```python
from build123d import *

# Parameters (mm, degrees)
SKETCH_1_R          = 2
EXTRUDE_1_DEPTH     = 10
SKETCH_2_R          = 1.5
CUT_EXTRUDE_1_DEPTH = 6
SKETCH_3_W          = 5
SKETCH_3_H          = 9
CUT_EXTRUDE_2_DEPTH = 13


with BuildPart() as part:
    # 草图1 → 凸台-拉伸1 (new body)
    with BuildSketch(Plane.XY):
        with BuildLine():
            Line((-46.664590164, 1.25102459), (-27.024590164, 1.25102459))
            Line((-27.024590164, 1.25102459), (-27.024590164, 6.25102459))
            Line((-27.024590164, 6.25102459), (0.975409836, 6.25102459))
            Line((0.975409836, 6.25102459), (0.975409836, 10.25102459))
            Line((0.975409836, 10.25102459), (6.975409836, 10.25102459))
            Line((6.975409836, 10.25102459), (6.975409836, -12.74897541))
            Line((6.975409836, -12.74897541), (-54.524590164, -12.74897541))
            Line((-54.524590164, -12.74897541), (-54.524590164, 1.25102459))
            ThreePointArc((-54.524590164, 1.25102459), (-53.342455561, 3.873523399), (-50.594590164, 4.724509872))
            ThreePointArc((-50.594590164, 4.724509872), (-47.846724767, 3.873523399), (-46.664590164, 1.25102459))
        make_face()
        with Locations((-51.024590164, 1.25102459)):
            Circle(SKETCH_1_R, mode=Mode.SUBTRACT)
    extrude(amount=EXTRUDE_1_DEPTH)

    # 草图2 → 切除-拉伸1 (cut)
    with BuildSketch(Plane(origin=(6.975409836, 0, 0), x_dir=(0, 0, -1), z_dir=(1, 0, 0))):
        with Locations((-5, 7.25102459)):
            Circle(SKETCH_2_R)
    extrude(amount=-CUT_EXTRUDE_1_DEPTH, mode=Mode.SUBTRACT)

    # 草图3 → 切除-拉伸2 (cut)
    with BuildSketch(Plane.ZY.offset(54.524590164)):
        with Locations((5, 0.25102459)):
            Rectangle(SKETCH_3_W, SKETCH_3_H)
    extrude(amount=-CUT_EXTRUDE_2_DEPTH, mode=Mode.SUBTRACT)


solid = part.part
```
The listing builds one solid part. Answer for the finished solid, in the listing's coordinates (mm). A direction names the side the tool comes from. Coordinates: 2 decimals unless noted, no trailing zeros. Order: outer loops, then holes, each group sorted by start corner. A loop starts at its lowest first (then second) coordinate and runs counter-clockwise, first axis right, second up. Notation, with made-up numbers: M -4.5,41.5 L 11.5,41.5 A16 cw 11.5,50.5 Z; hole C 69,-10.75 d8. An arc over 180 degrees is marked long. Answer as a JSON object with one key per item and string values. Group by question number.
1. Section D-D on z = 1.75 is taken. Write down the section's boundary in (x, y), then the cut area to 3 significant figures.
2. Determine the mould class of faces 1 (the flat face through (0.975, 9, 5)), 2 (the cylindrical face through (-49.177, 0.485, 1.232)), 3 (the cylindrical face through (-49.177, 0.485, 8.732)), 4 (the flat face through (-48, -4.249, 5)) for opening direction X: released by +X, released by -X, zero draft, split by the parting line, or undercut.
3. Straight lines are drawn through the part: line 1 (Y direction, x = 4.1, z = 5); line 2 (Y direction, x = -1, z = 9.5); line 3 (X direction, y = 8.75, z = 8). For each, find the intervals that lie inside material, in ascending order.
4. Section B-B on y = 0.5 is taken. Write down the section's boundary in (x, z), then the cut area to 3 significant figures.
5. Section C-C on x = -29.5 is taken. Write down the section's boundary in (y, z), then the cut area to 3 significant figures.
6. Flat-ended cylindrical pins translate along their axes: P1, Ø6, axis at x = -18.5, z = 7, coming from the +Y side; P2, Ø2.5, axis at y = 3.5, z = 7.5, coming from the -X side; P3, Ø2, axis at y = 9, z = 5, coming from the -X side. Find the tip coordinate at first contact, or state that the pin passes through.
7. Section A-A on z = 5 is taken. Write down the section's boundary in (x, y), then the cut area to 4 significant figures.
8. A tool of negligible diameter and unlimited length cuts with its end or side. For faces 5 (the cylindrical face through (4.017, 5.787, 5.325)), 6 (the flat face through (-48, -1, 2.5)), 7 (the flat face through (-37, 1.251, 5)), 8 (the flat face through (-13, 6.251, 5)), from which of +Z, -Z, +X, -X, +Y, -Y can it reach the whole face along a straight path? Write none if from no direction.
Values follow:
{
 "1": {"outline": "M -54.52,-12.75 L 6.98,-12.75 L 6.98,10.25 L 0.98,10.25 L 0.98,6.25 L -27.02,6.25 L -27.02,1.25 L -46.66,1.25 A3.5 ccw -50.59,4.72 A3.5 ccw -54.52,1.25 Z; hole C -51.02,1.25 d4", "area": "1,060 mm2"},
 "2": {"face 1": "released by -X", "face 2": "undercut", "face 3": "undercut", "face 4": "zero draft"},
 "3": {"line 1": "-12.75 to 5.75, 8.75 to 10.25", "line 2": "-12.75 to 6.25", "line 3": "0.98 to 6.98"},
 "4": {"outline": "M -54.52,0 L -52.88,0 L -52.88,2.5 L -54.52,2.5 Z; M -54.52,7.5 L -52.88,7.5 L -52.88,10 L -54.52,10 Z; M -49.17,0 L 6.98,0 L 6.98,10 L -49.17,10 L -49.17,7.5 L -41.52,7.5 L -41.52,2.5 L -49.17,2.5 Z", "area": "531 mm2"},
 "5": {"outline": "M -12.75,0 L 1.25,0 L 1.25,10 L -12.75,10 Z", "area": "140 mm2"},
 "6": {"P1": "y = 6.25", "P2": "x = -54.38", "P3": "x = 0.98"},
 "7": {"outline": "M -54.52,-12.75 L 6.98,-12.75 L 6.98,5.75 L 0.98,5.75 L 0.98,6.25 L -27.02,6.25 L -27.02,1.25 L -41.52,1.25 L -41.52,-4.25 L -54.52,-4.25 Z; M 0.98,8.75 L 6.98,8.75 L 6.98,10.25 L 0.98,10.25 Z", "area": "965.5 mm2"},
 "8": {"face 5": "+X", "face 6": "-X, +Y", "face 7": "+Z, -Z, +Y", "face 8": "+Z, -Z, -X, +Y"}
}
